from build123d import *

# Parameters (mm, degrees)
SKETCH_1_R      = 31.5
EXTRUDE_1_DEPTH = 10
SKETCH_2_R      = 20
EXTRUDE_2_DEPTH = 400
SKETCH_3_R      = 18
EXTRUDE_3_DEPTH = 39
FILLET_1_R      = 2
CHAMFER_2_SIZE  = 1
CHAMFER_3_SIZE  = 0.5


with BuildPart() as part:
    # 草图1 → 凸台-拉伸1 (new body)
    with BuildSketch(Plane.XY):
        Circle(SKETCH_1_R)
    extrude(amount=EXTRUDE_1_DEPTH)

    # 草图2 → 凸台-拉伸2 (add)
    with BuildSketch(Plane.XY.offset(10)):
        Circle(SKETCH_2_R)
    extrude(amount=EXTRUDE_2_DEPTH)

    # 草图3 → 凸台-拉伸3 (add)
    with BuildSketch(Plane.XY.offset(410)):
        Circle(SKETCH_3_R)
    extrude(amount=EXTRUDE_3_DEPTH)

    # 圆角1
    fillet_1_edges = [part.edges().sort_by_distance(p)[0] for p in [
        (-20, 0, 10),
    ]]
    fillet(fillet_1_edges, radius=FILLET_1_R)

    # 倒角2
    chamfer_2_edges = [part.edges().sort_by_distance(p)[0] for p in [
        (-18, 0, 449),
        (-20, 0, 410),
    ]]
    chamfer(chamfer_2_edges, length=CHAMFER_2_SIZE)

    # 倒角3
    chamfer_3_edges = [part.edges().sort_by_distance(p)[0] for p in [
        (-31.5, 0, 0),
        (-31.5, 0, 10),
    ]]
    chamfer(chamfer_3_edges, length=CHAMFER_3_SIZE)


solid = part.part
Could you check a few things on this model? Use its own coordinates, in mm. A direction names the side the tool comes from. Give positions to 0.01 mm unless a question says otherwise; leave off trailing zeros. Order: outer loops, then holes, each group sorted by start corner. A loop starts at its lowest first (then second) coordinate and runs counter-clockwise, first axis right, second up. Notation, with made-up numbers: (88.25, 60) - (108.25, 60) arc R21 ccw to (108.25, 96) - close; hole circle Ø3 at (5, 34.25). An arc over 180 degrees is marked (long way). One line per item, written item: value. Start each with the question number.
1. Imagine slicing it at C-C on z = 304.5. List the corners of the cut face in (x, y) for me, plus the area to 3 significant figures.
2. If I drill on probe 1 along X at (y, z) = (6, 39.5); probe 2 along Z at (x, y) = (-25, -3.5); probe 3 along Y at (x, z) = (10.5, 53.5), over which ranges is the centre line in solid material (lowest first)?
3. For P1, Ø5, axis at y = -19.5, z = 277, coming from the -X side; P2, Ø8, axis at x = 8.5, z = 212.5, coming from the +Y side; P3, Ø10, axis at y = -18, z = 303, coming from the +X side, each with a flat end and sliding along its axis, tell me the tip position at first contact or that it passes through.
4. Imagine slicing it at A-A on y = 0. List the corners of the cut face in (x, z) for me.
5. For faces 1 (the face through (-4.336, -19.524, 207.721)), 2 (the face through (0, 0, 449)), which set-ups out of +Z, -Z, +X, -X, +Y, -Y let a thin tool reach every point of the face, with its end or its side?
Values:
1. outline: circle Ø40 at (0, 0)
1. area: 1,260 mm²
2. probe 1: -19.08 to 19.08
2. probe 2: 0 to 10
2. probe 3: -17.02 to 17.02
3. P1: x = -10.54
3. P2: y = 19.49
3. P3: x = 15.2
4. outline: (-31.5, 0.5) - (-31, 0) - (31, 0) - (31.5, 0.5) - (31.5, 9.5) - (31, 10) - (22, 10) arc R2 cw to (20, 12) - (20, 409) - (19, 410) - (18, 410) - (18, 448) - (17, 449) - (-17, 449) - (-18, 448) - (-18, 410) - (-19, 410) - (-20, 409) - (-20, 12) arc R2 cw to (-22, 10) - (-31, 10) - (-31.5, 9.5) - close
5. face 1: +Z
5. face 2: +Z, +X, -X, +Y, -Y
